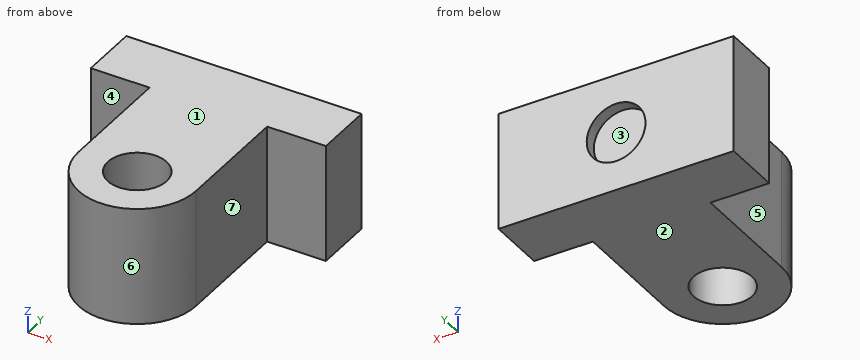
from build123d import *

# Parameters (mm, degrees)
SKETCH1_R           = 2.5
BOSS_EXTRUDE1_DEPTH = 10
SKETCH2_R           = 2.5
CUT_EXTRUDE1_DEPTH  = 1


with BuildPart() as part:
    # Sketch1 → Boss-Extrude1 (new body)
    with BuildSketch(Plane.XY):
        with BuildLine():
            Line((-5, 0), (-5, 10))
            Line((-5, 10), (-10, 10))
            Line((-10, 10), (-10, 15))
            Line((-10, 15), (10, 15))
            Line((10, 15), (10, 10))
            Line((10, 10), (5, 10))
            Line((5, 10), (5, 0))
            ThreePointArc((5, 0), (0, -5), (-5, 0))
        make_face()
        Circle(SKETCH1_R, mode=Mode.SUBTRACT)
    extrude(amount=BOSS_EXTRUDE1_DEPTH)

    # Sketch2 → Cut-Extrude1 (cut)
    with BuildSketch(Plane(origin=(0, 15, 0), x_dir=(1, 0, 0), z_dir=(0, 1, 0))):
        with Locations(Location((0, -5, 0), (0, 0, 270))):
            Circle(SKETCH2_R)
    extrude(amount=-CUT_EXTRUDE1_DEPTH, mode=Mode.SUBTRACT)


solid = part.part
Geometry: final body of the model. Coordinates: model frame, mm. Face numbers are marked on the shaded views. A direction names the side the tool comes from. Coordinates: 2 decimals unless noted, no trailing zeros. Order: outer loops, then holes, each group sorted by start corner. A loop starts at its lowest first (then second) coordinate and runs counter-clockwise, first axis right, second up.
1) Set-up query: the marked faces 5, 6 and 7. Return all of +Z, -Z, +X, -X, +Y, -Y with unobstructed straight access to the full face (end or side cutting, diameter ignored); none if empty.
Result sheet:
face 5: +Z, -Z, -X, -Y
face 6: +Z, -Z, -Y
face 7: +Z, -Z, +X, -Y
2) Section D-D (z = 5). Return loops of the section in (x, y).
Result sheet:
outline: (-10, 10) - (-5, 10) - (-5, 0) arc R5 ccw to (5, 0) - (5, 10) - (10, 10) - (10, 15) - (2.5, 15) - (2.5, 14) - (-2.5, 14) - (-2.5, 15) - (-10, 15) - close; hole circle Ø5 at (0, 0)
3) Section A-A (z = 2.25). Return loops of the section in (x, y), then the cut area to 3 significant figures.
Result sheet:
outline: (-10, 10) - (-5, 10) - (-5, 0) arc R5 ccw to (5, 0) - (5, 10) - (10, 10) - (10, 15) - (-10, 15) - close; hole circle Ø5 at (0, 0)
area: 220 mm2
4) Section B-B (x = 0). Return loops of the section in (y, z), then the cut area to 3 significant figures.
Result sheet:
outline: (-5, 0) - (-2.5, 0) - (-2.5, 10) - (-5, 10) - close; (2.5, 0) - (15, 0) - (15, 2.5) - (14, 2.5) - (14, 7.5) - (15, 7.5) - (15, 10) - (2.5, 10) - close
area: 145 mm2
5) Section C-C (y = -1). Return loops of the section in (x, z), then the cut area to 3 significant figures.
Result sheet:
outline: (-4.9, 0) - (-2.29, 0) - (-2.29, 10) - (-4.9, 10) - close; (2.29, 0) - (4.9, 0) - (4.9, 10) - (2.29, 10) - close
area: 52.2 mm2
6) First-contact query: P1, Ø3, axis at y = -1.5, z = 4.5, coming from the +X side; P2, Ø5.5, axis at x = -8, z = 7.5, coming from the -Y side; P3, Ø6, axis at y = -2.5, z = 3.5, coming from the -X side; P4, Ø4.5, axis at x = 0, y = 0, coming from the -Z side. Flat tips, straight axial feed; report the tip coordinate or a pass-through.
Result sheet:
P1: stops at x = 5
P2: stops at y = 10
P3: stops at x = -5
P4: passes through
7) Ray query, probe 1 along Y at (x, z) = (0, 3); probe 2 along X at (y, z) = (14.6, 5); probe 3 along X at (y, z) = (5.5, 1.5). Return the intervals inside material, ascending.
Result sheet:
probe 1: y = -5 to -2.5, 2.5 to 14
probe 2: x = -10 to -2.5, 2.5 to 10
probe 3: x = -5 to 5
8) Draft query along Z for the marked faces 1, 2, 3 and 4. Return one class per face: released by +Z, released by -Z, zero draft, split by the parting line, or undercut.
Result sheet:
face 1: released by +Z
face 2: released by -Z
face 3: undercut
face 4: zero draft
